from build123d import *

# Parameters (mm, degrees)
ARM_BODY_DEPTH          = 24
BUSHING_BOSS_SKETCH_R   = 16
BUSHING_BOSS_SKETCH_R_2 = 8
BUSHING_BOSS_32_DEPTH   = 40
PIVOT_LUG_SKETCH_R      = 28
PIVOT_LUG_56_DEPTH      = 34
CLEVIS_SLOT_SKETCH_W    = 56
CLEVIS_SLOT_SKETCH_H    = 16
CLEVIS_SLOT_16MM_DEPTH  = 170.198108736
PIVOT_BORE_30_D         = 30


with BuildPart() as part:
    # Arm Profile Sketch → Arm Body (new, symmetric)
    with BuildSketch(Plane.XY):
        with BuildLine():
            Line((0, 0), (28, 0))
            Line((28, 0), (28, 8))
            ThreePointArc((28, 8), (30.343145751, 13.656854249), (36, 16))
            Line((36, 16), (76, 16))
            ThreePointArc((76, 16), (81.656854249, 13.656854249), (84, 8))
            Line((84, 8), (84, -24))
            Line((84, -24), (128, -24))
            Line((128, -24), (128, 32))
            Line((128, 32), (56, 32))
            ThreePointArc((56, 32), (50.343145751, 34.343145751), (48, 40))
            Line((48, 40), (0, 40))
            Line((0, 40), (0, 0))
        make_face()
    extrude(amount=ARM_BODY_DEPTH, both=True)

    # Bushing Boss Sketch → Bushing Boss Ø32 (add)
    with BuildSketch(Plane(origin=(0, 40, 0), x_dir=(1, 0, 0), z_dir=(0, 1, 0))):
        with Locations((24, 0)):
            Circle(BUSHING_BOSS_SKETCH_R)
        with Locations(Location((24, 0, 0), (0, 0, 180))):
            Circle(BUSHING_BOSS_SKETCH_R_2, mode=Mode.SUBTRACT)
    extrude(amount=BUSHING_BOSS_32_DEPTH)

    # Pivot Lug Sketch → Pivot Lug Ø56 (add, symmetric)
    with BuildSketch(Plane.XY):
        with Locations((128, 4)):
            Circle(PIVOT_LUG_SKETCH_R)
    extrude(amount=PIVOT_LUG_56_DEPTH, both=True)

    # Clevis Slot Sketch → Clevis Slot 16mm (cut, through all)
    with BuildSketch(Plane(origin=(0, 32, 0), x_dir=(1, 0, 0), z_dir=(0, 1, 0))):
        with Locations((128, 0)):
            Rectangle(CLEVIS_SLOT_SKETCH_W, CLEVIS_SLOT_SKETCH_H)
    extrude(amount=-CLEVIS_SLOT_16MM_DEPTH, mode=Mode.SUBTRACT)

    # Pivot Bore Ø30 (through all)
    with Locations(Plane.XY.offset(34)):
        with Locations((128, 4)):
            Hole(PIVOT_BORE_30_D / 2)


solid = part.part
Check sheet for the modelled part. Datum: model origin and axes. Units: mm. A direction names the side the tool comes from. Round coordinates to 2 decimals unless told otherwise and drop trailing zeros. Order: outer loops, then holes, each group sorted by start corner. A loop starts at its lowest first (then second) coordinate and runs counter-clockwise, first axis right, second up.
(1) Scan lines: probe 1 along X at (y, z) = (0.5, -12); probe 2 along Z at (x, y) = (119.5, 26.5); probe 3 along Z at (x, y) = (24, 55). Record each from-to range of solid material in increasing order.
(2) Cross-section at A-A, the plane y = 4. Enter the section's corners in (x, z).
(3) Cross-section at C-C, the plane z = 0. Enter the section's corners in (x, y), and give its area (3 significant figures).
(4) Draft check along Y on faces 1 (the flat face through (24, 40, 0)), 2 (the cylindrical face through (142.985, 4.66, -21.182)), 3 (the flat face through (96, -24, 0)), 4 (the cylindrical face through (30.349, 59.72, -4.868)). Enter one of: pulls with the +Y half, pulls with the -Y half, needs draft (parallel to the pull), parting line crosses it, or undercut.
(5) Cross-section at B-B, the plane x = 109. Enter the section's corners in (y, z), and give its area (3 significant figures).
(6) Go/stop test with flat-tipped pins: P1, Ø22.5, axis at x = 15, z = 10, coming from the -Y side; P2, Ø8, axis at y = 13.5, z = 0.5, coming from the +X side; P3, Ø8, axis at x = 25.5, z = -2.5, coming from the +Y side. Record where each tip stops, or that it passes through.
(7) Cross-section at D-D, the plane x = 24. Enter the section's corners in (y, z), and give its area (3 significant figures).
(8) Access from +Z, -Z, +X, -X, +Y, -Y to the whole of each face (thin tool, end or side, straight path). Record for faces 5 (the flat face through (40.3, 40, 0.3)), 6 (the flat face through (14, 0, 0)), 7 (the cylindrical face through (154.707, 12.41, 24.071)), 8 (the flat face through (115, -8, -8)), 9 (the cylindrical face through (30.281, 13.594, 0.336)).
Check sheet entries:
1. probe 1: x = 0 to 28, 84 to 113.41, 142.59 to 155.78
1. probe 2: z = -34 to -8, 8 to 34
1. probe 3: z = -16 to -8, 8 to 16
2. outline: (0, -24) - (28, -24) - (28, 24) - (0, 24) - close; (84, -24) - (100, -24) - (100, -34) - (113, -34) - (113, -8) - (100, -8) - (100, 8) - (113, 8) - (113, 34) - (100, 34) - (100, 24) - (84, 24) - close; (143, -34) - (156, -34) - (156, -8) - (143, -8) - close; (143, 8) - (156, 8) - (156, 34) - (143, 34) - close
3. outline: (0, 0) - (28, 0) - (28, 8) arc R8 cw to (36, 16) - (76, 16) arc R8 cw to (84, 8) - (84, -24) - (100, -24) - (100, 32) - (56, 32) arc R8 cw to (48, 40) - (40, 40) - (40, 80) - (32, 80) - (32, 40) - (16, 40) - (16, 80) - (8, 80) - (8, 40) - (0, 40) - close
3. area: 3,750 mm2
4. face 1: pulls with the +Y half
4. face 2: undercut
4. face 3: pulls with the -Y half
4. face 4: needs draft
5. outline: (-24, -24) - (-16.57, -24) - (-16.57, -34) - (24.57, -34) - (24.57, -24) - (32, -24) - (32, -8) - (-24, -8) - close; (-24, 8) - (32, 8) - (32, 24) - (24.57, 24) - (24.57, 34) - (-16.57, 34) - (-16.57, 24) - (-24, 24) - close
5. area: 2,610 mm2
6. P1: stops at y = 0
6. P2: stops at x = 100
6. P3: stops at y = 40
7. outline: (0, -24) - (40, -24) - (40, -16) - (80, -16) - (80, -8) - (40, -8) - (40, 8) - (80, 8) - (80, 16) - (40, 16) - (40, 24) - (0, 24) - close
7. area: 2,560 mm2
8. face 5: +Y
8. face 6: +Z, -Z, -X, -Y
8. face 7: +Z
8. face 8: +X, +Y, -Y
8. face 9: +Z, -Z, -Y
